```python
from build123d import *

# Parameters (mm, degrees)
CLEVIS_BODY_DEPTH    = 22.5
CROSS_HOLE_SKETCH_R  = 6
CROSS_HOLE_DEPTH     = 84
COUNTERBORE_SKETCH_R = 12
COUNTERBORE_24_DEPTH = 9
MOUNTING_START       = -22.5
MOUNTING_TAB_DEPTH   = 4.5
ANGLED_LIP_DEPTH     = 60
RELIEF_CUT_DEPTH     = 9
TAB_SLOT_SKETCH_R    = 7.5
TAB_SLOT_DEPTH       = 9


with BuildPart() as part:
    # Clevis Body Sketch → Clevis Body (new, symmetric)
    with BuildSketch(Plane(origin=(0, 0, 0), x_dir=(1, 0, 0), z_dir=(0, 1, 0))):
        with BuildLine():
            Line((-12, 9), (-60, 9))
            Line((-60, 9), (-60, 30))
            Line((-60, 30), (0, 30))
            ThreePointArc((0, 30), (30, 0), (0, -30))
            Line((0, -30), (-60, -30))
            Line((-60, -30), (-60, -9))
            Line((-60, -9), (-12, -9))
            ThreePointArc((-12, -9), (15, 0), (-12, 9))
        make_face()
    extrude(amount=CLEVIS_BODY_DEPTH, both=True)

    # Cross Hole Sketch → Cross Hole (cut)
    with BuildSketch(Plane.XY.offset(30)):
        with Locations((-36, 0)):
            Circle(CROSS_HOLE_SKETCH_R)
    extrude(amount=-CROSS_HOLE_DEPTH, mode=Mode.SUBTRACT)

    # Counterbore Sketch → Counterbore Ø24 (cut)
    with BuildSketch(Plane.XY.offset(30)):
        with Locations((-36, 0)):
            Circle(COUNTERBORE_SKETCH_R)
    counterbore_24 = extrude(amount=-COUNTERBORE_24_DEPTH, mode=Mode.SUBTRACT)

    # Counterbore Mirror: Counterbore Ø24 across plane
    add(counterbore_24.mirror(Plane.XY), mode=Mode.SUBTRACT)

    # Mounting Tab Sketch → Mounting Tab (add, symmetric)
    with BuildSketch(Plane(origin=(0, 22.5, 0), x_dir=(1, 0, 0), z_dir=(0, 1, 0)).offset(MOUNTING_START)):
        with BuildLine():
            Line((0, 30), (90, 30))
            Line((90, 30), (90, -30))
            Line((90, -30), (0, -30))
            ThreePointArc((0, -30), (30, 0), (0, 30))
        make_face()
    extrude(amount=MOUNTING_TAB_DEPTH, both=True)

    # Angled Lip Sketch → Angled Lip (add)
    with BuildSketch(Plane.XY.offset(30)):
        Polygon((90, -4.5), (90, 4.5), (132.779960262, 47.279960262), (139.143921292, 40.915999231), align=None)
    extrude(amount=-ANGLED_LIP_DEPTH)

    # Relief Cut Sketch → Relief Cut (cut)
    with BuildSketch(Plane(origin=(0, 4.5, 0), x_dir=(1, 0, 0), z_dir=(0, 1, 0))):
        with BuildLine():
            Line((51, -30), (51, 0))
            ThreePointArc((51, 0), (60, 9), (69, 0))
            Line((69, 0), (69, -30))
            Line((69, -30), (51, -30))
        make_face()
    extrude(amount=-RELIEF_CUT_DEPTH, mode=Mode.SUBTRACT)

    # Tab Slot Sketch → Tab Slot (cut)
    with BuildSketch(Plane(origin=(42.75, -42.75, 0), x_dir=(0, 0, 1), z_dir=(-0.7071067811865488, 0.7071067811865464, 0))):
        with Locations(Location((0, 104.821590822, 0), (0, 0, 270))):
            Circle(TAB_SLOT_SKETCH_R)
        with BuildLine():
            Line((-30, 66.821590822), (-14.073626439, 110.011295906))
            ThreePointArc((-14.073626439, 110.011295906), (0, 119.821590822), (14.073626439, 110.011295906))
            Line((14.073626439, 110.011295906), (30, 66.821590822))
            Line((30, 66.821590822), (30, 127.321590822))
            Line((30, 127.321590822), (-30, 127.321590822))
            Line((-30, 127.321590822), (-30, 66.821590822))
        make_face()
    extrude(amount=-TAB_SLOT_DEPTH, mode=Mode.SUBTRACT)


solid = part.part
```
Geometry check sheet. Reference: the model listing, model coordinates, mm. A direction names the side the tool comes from. Coordinates: 2 decimals unless noted, no trailing zeros. Order: outer loops, then holes, each group sorted by start corner. A loop starts at its lowest first (then second) coordinate and runs counter-clockwise, first axis right, second up. Notation, with made-up numbers: (67.25, -20.75) - (74.25, -20.75) arc R14 ccw to (74.25, 6.25) - close; hole circle Ø7 at (31, 79). An arc over 180 degrees is marked (long way). Answer as a JSON object with one key per item and string values. Group by question number.
Item 1: Depth check by flat-ended pin: pin 1 Ø7 at (y, z) = (-2, 12) entering from +X; pin 2 Ø5 at (x, z) = (84, 6) entering from +Y; pin 3 Ø4 at (x, z) = (13.5, -15.5) entering from +Y; pin 4 Ø11 at (x, y) = (-36, 0) entering from +Z. Enter the tip coordinate at first touch or a pass-through.
Item 2: Sectioned sample at C-C, the plane y = 16. Record the cut outline in (x, z), and give its area (3 significant figures).
Item 3: Tool access check on faces 1 (the face through (104.3, 18.8, 0.4)), 2 (the face through (-14, 22.5, -14)), 3 (the face through (51, 0, 15)), 4 (the face through (-31, 5, 9)), 5 (the face through (-34, 6, -21)). Record the directions out of +Z, -Z, +X, -X, +Y, -Y that give a thin tool (end or side, any length) a straight path to the whole face; none if there is none.
Item 4: Sectioned sample at A-A, the plane x = -36. Record the cut outline in (y, z).
Item 5: Sectioned sample at D-D, the plane y = -14.5. Record the cut outline in (x, z).
Item 6: Draft check along Z on faces 6 (the face through (60, 0, -9)), 7 (the face through (-30, 5, -9)), 8 (the face through (69, 0, 15)). Enter one of: +Z half, -Z half, draft (parallel to the pull), parting line (faces both ways), or undercut.
Item 7: Sectioned sample at B-B, the plane z = 17.5. Record the cut outline in (x, y), and give its area (3 significant figures).
Item 8: Scan lines: probe 1 along Y at (x, z) = (-36, -24.75); probe 2 along Z at (x, y) = (-16.5, -19); probe 3 along Y at (x, z) = (-36, 12). Record each from-to range of solid material in increasing order.
Resolved:
{
 "1": {"pin 1": "x = 96.49", "pin 2": "y = 4.5", "pin 3": "y = 22.5", "pin 4": "through"},
 "2": {"outline": "(-60, -30) - (0, -30) arc R30 ccw to (0, 30) - (-60, 30) - (-60, 9) - (-12, 9) arc R15 cw (long way) to (-12, -9) - (-60, -9) - close; (101.5, -24) - (112.18, -21.22) - (112.18, 21.22) - (101.5, 24) - close", "area": "3,960 mm^2"},
 "3": {"face 1": "+Z, -Z, +Y", "face 2": "+Z, -Z, -X, +Y", "face 3": "+Z, +Y, -Y", "face 4": "-X, +Y, -Y", "face 5": "-Z"},
 "4": {"outline": "(-22.5, -30) - (-12, -30) - (-12, -21) - (-6, -21) - (-6, -9) - (-22.5, -9) - close; (-22.5, 9) - (-6, 9) - (-6, 21) - (-12, 21) - (-12, 30) - (-22.5, 30) - close; (6, -21) - (12, -21) - (12, -30) - (22.5, -30) - (22.5, -9) - (6, -9) - close; (6, 9) - (22.5, 9) - (22.5, 30) - (12, 30) - (12, 21) - (6, 21) - close"},
 "5": {"outline": "(-60, -30) - (0, -30) arc R30 ccw to (0, 30) - (-60, 30) - (-60, 9) - (-12, 9) arc R15 cw (long way) to (-12, -9) - (-60, -9) - close"},
 "6": {"face 6": "+Z half", "face 7": "undercut", "face 8": "draft"},
 "7": {"outline": "(-60, -22.5) - (24.37, -22.5) - (24.37, -4.5) - (51, -4.5) - (51, 4.5) - (24.37, 4.5) - (24.37, 22.5) - (-60, 22.5) - close; (69, -4.5) - (90, -4.5) - (119.59, 22.85) - (113.97, 28.47) - (90, 4.5) - (69, 4.5) - close; hole circle Ø12 at (-36, 0)", "area": "4,380 mm^2"},
 "8": {"probe 1": "-22.5 to -12, 12 to 22.5", "probe 2": "-30 to -9, 9 to 30", "probe 3": "-22.5 to -6, 6 to 22.5"}
}
